from build123d import *

# Parameters (mm, degrees)
SKETCH_2_R          = 35
EXTRUDE_1_DEPTH     = 12
SKETCH_3_R          = 2.25
CUT_EXTRUDE_1_DEPTH = 51.931326313


with BuildPart() as part:
    # 草图2 → 凸台-拉伸1 (new body)
    with BuildSketch(Plane.XY):
        Circle(SKETCH_2_R)
        with BuildLine():
            ThreePointArc((-12.484738743, -24.502679415), (-20.031862375, -18.840766699), (-25.22108467, -10.961153593))
            ThreePointArc((-25.22108467, -10.961153593), (-25.259217651, 8.481414129), (-11.122767244, 21.829659843))
            ThreePointArc((-11.122767244, 21.829659843), (8.485416214, 24.001994273), (24.502679415, 12.484738743))
            ThreePointArc((24.502679415, 12.484738743), (26.716793299, 6.418124257), (26, 0))
            ThreePointArc((26, 0), (24.576877243, -5.809609847), (21.829659843, -11.122767244))
            ThreePointArc((21.829659843, -11.122767244), (9.253297944, -24.916386782), (-9.389722524, -25.847303746))
            ThreePointArc((-9.389722524, -25.847303746), (-10.960408212, -25.228341041), (-12.484738743, -24.502679415))
        make_face(mode=Mode.SUBTRACT)
    extrude(amount=EXTRUDE_1_DEPTH)

    # 草图3 → 切除-拉伸1 (cut, through all)
    with BuildSketch(Plane.XY.offset(12)):
        with Locations((0, 31)):
            Circle(SKETCH_3_R)
        with Locations((30.917947145, 0.049389692)):
            Circle(SKETCH_3_R)
        with Locations((-0.047414981, -30.978569044)):
            Circle(SKETCH_3_R)
        with Locations((-31.016726529, -0.148169076)):
            Circle(SKETCH_3_R)
    extrude(amount=-CUT_EXTRUDE_1_DEPTH, mode=Mode.SUBTRACT)


solid = part.part
Design review of the part built by this model. Coordinates are the model's own, in mm. A direction names the side the tool comes from. Coordinates: 2 decimals unless noted, no trailing zeros. Order: outer loops, then holes, each group sorted by start corner. A loop starts at its lowest first (then second) coordinate and runs counter-clockwise, first axis right, second up.
Item 1: Take a section at C-C, the plane y = 31. Write out the cut boundary in (x, z), then the cut area to 3 significant figures.
Item 2: For faces 1 (the cylindrical face through (-25.37, 8.22, 5.92)), 2 (the flat face through (-7.9, 23.5, 0)), list the 3-axis set-ups (+Z, -Z, +X, -X, +Y, -Y) from which the entire face can be reached by the end or side of a thin tool; tool diameter is ignored.
Item 3: The part is to be moulded in two halves that separate along X. For faces 3 (the cylindrical face through (-28, -21, 6)), 4 (the cylindrical face through (-19.94, -18.94, 5.92)), 5 (the flat face through (-7.9, 23.5, 12)), say which applies: pulls with the +X half, pulls with the -X half, needs draft (parallel to the pull), parting line crosses it, or undercut.
Item 4: For line 1 (X direction, y = -1, z = 1.5); line 2 (Y direction, x = 17, z = 9.25); line 3 (X direction, y = 17.5, z = 2), list the stretches that pass through material, from the lowest coordinate up.
Item 5: For pin 1 Ø8 at (x, y) = (28, 11) entering from -Z; pin 2 Ø1 at (x, z) = (-25.5, 10.5) entering from -Y; pin 3 Ø6 at (x, y) = (-4.5, 18.5) entering from +Z; pin 4 Ø1.5 at (y, z) = (3.5, 1.5) entering from +X, all flat-tipped, find the tip position at first contact; note any pin that passes through.
Item 6: Take a section at A-A, the plane x = -6. Write out the cut boundary in (y, z), then the cut area to 3 significant figures.
Item 7: Take a section at B-B, the plane z = 8.5. Write out the cut boundary in (x, y).
The answers:
1. outline: (-16.25, 0) - (-2.25, 0) - (-2.25, 12) - (-16.25, 12) - close; (2.25, 0) - (16.25, 0) - (16.25, 12) - (2.25, 12) - close
1. area: 336 mm2
2. face 1: +Z, -Z
2. face 2: -Z, +X, -X, +Y, -Y
3. face 3: parting line crosses it
3. face 4: undercut
3. face 5: needs draft
4. line 1: x = -34.99 to -33.1, -28.93 to -27.25, 25.86 to 28.93, 32.91 to 34.99
4. line 2: y = -30.59 to -19.16, 20.12 to 30.59
4. line 3: x = -30.31 to -18.59, 20.28 to 30.31
5. pin 1: stops at z = 0
5. pin 2: stops at y = -24.49
5. pin 3: passes through
5. pin 4: stops at x = 34.89
6. outline: (-34.48, 0) - (-26.78, 0) - (-26.78, 12) - (-34.48, 12) - close; (23.86, 0) - (34.48, 0) - (34.48, 12) - (23.86, 12) - close
6. area: 220 mm2
7. outline: circle Ø70 at (0, 0); hole circle Ø4.5 at (-31.02, -0.15); hole (-25.22, -10.96) arc R27.5 ccw to (-12.48, -24.5) arc R24.5 ccw to (21.83, -11.12) arc R25.3 ccw to (26, 0) arc R14.13 ccw to (24.5, 12.48) arc R27.5 ccw to (-11.12, 21.83) arc R24.5 ccw to start; hole circle Ø4.5 at (-0.05, -30.98); hole circle Ø4.5 at (0, 31); hole circle Ø4.5 at (30.92, 0.05)
